Model file for the job. Use its own axes, mm. A direction names the side the tool comes from. Round coordinates to 2 decimals unless told otherwise and drop trailing zeros. Loops run counter-clockwise (first coordinate to the right, second up) from the corner with the lowest first, then second, coordinate; pieces in that order, holes last. Notation, with made-up numbers: M 61.5,46 L 92.5,46 A22 cw 92.5,54 Z; hole C 18.25,12.5 d4. An arc over 180 degrees is marked long. Answer in a Markdown table with one row per item.
from build123d import *

# Parameters (mm, degrees)
SKETCH1_R           = 40
BOSS_EXTRUDE1_DEPTH = 33
CUT_EXTRUDE1_START  = -6
SKETCH2_R           = 40
SKETCH2_R_2         = 38
CUT_EXTRUDE1_DEPTH  = 6
CHAMFER1_SIZE       = 5
SKETCH3_R           = 14
CUT_EXTRUDE2_DEPTH  = 13
CUT_EXTRUDE3_DEPTH  = 20


with BuildPart() as part:
    # Sketch1 → Boss-Extrude1 (new body)
    with BuildSketch(Plane.XY):
        Circle(SKETCH1_R)
    extrude(amount=BOSS_EXTRUDE1_DEPTH)

    # Sketch2 → Cut-Extrude1 (cut)
    with BuildSketch(Plane.XY.offset(33).offset(CUT_EXTRUDE1_START)):
        Circle(SKETCH2_R)
        Circle(SKETCH2_R_2, mode=Mode.SUBTRACT)
    extrude(amount=CUT_EXTRUDE1_DEPTH, mode=Mode.SUBTRACT)

    # Chamfer1
    chamfer1_edges = [part.edges().sort_by_distance(p)[0] for p in [
        (-40, 0, 0),
    ]]
    chamfer(chamfer1_edges, length=CHAMFER1_SIZE)

    # Sketch3 → Cut-Extrude2 (cut)
    with BuildSketch(Plane.XY.offset(33)):
        Circle(SKETCH3_R)
    extrude(amount=-CUT_EXTRUDE2_DEPTH, mode=Mode.SUBTRACT)

    # Sketch4 → Cut-Extrude3 (cut)
    with BuildSketch(Plane(origin=(0, 0, 0), x_dir=(-1, 0, 0), z_dir=(0, 0, -1))):
        Polygon((-19.5, -11.258330249), (0, -22.516660498), (19.5, -11.258330249), (19.5, 11.258330249), (0, 22.516660498), (-19.5, 11.258330249), align=None)
    extrude(amount=-CUT_EXTRUDE3_DEPTH, mode=Mode.SUBTRACT)


solid = part.part
1. Mould opens along X. For faces 4 (the flat face through (0, -15, 20)), 5 (the flat face through (35.4, -14.6, 27)), 6 (the cylindrical face through (12.932, -5.362, 26.591)), 7 (the cylindrical face through (-8.67, -39.05, 15.85)) say: +X half, -X half, draft (parallel to the pull), parting line (faces both ways), or undercut.
Verdict:
| item | result |
|---|---|
| face 4 | undercut |
| face 5 | draft |
| face 6 | undercut |
| face 7 | parting line |
2. Wall check: probe 1 along Y at (x, z) = (0, 26); probe 2 along X at (y, z) = (-21, 16); probe 3 along Y at (x, z) = (7.5, 13). Give the ranges that are in metal, low to high.
Verdict:
| item | result |
|---|---|
| probe 1 | y = -40 to -14, 14 to 40 |
| probe 2 | x = -34.04 to -2.63, 2.63 to 34.04 |
| probe 3 | y = -39.29 to -18.19, 18.19 to 39.29 |
3. Saw through at B-B (y = 0). Write the cut outline in (x, z), and give its area (3 significant figures).
Verdict:
| item | result |
|---|---|
| outline | M -40,5 L -35,0 L -19.5,0 L -19.5,20 L -14,20 L -14,33 L -38,33 L -38,27 L -40,27 Z; M 14,20 L 19.5,20 L 19.5,0 L 35,0 L 40,5 L 40,27 L 38,27 L 38,33 L 14,33 Z |
| area | 1,450 mm² |
4. Saw through at A-A (z = 7.5). Write the cut outline in (x, y).
Verdict:
| item | result |
|---|---|
| outline | C 0,0 d80; hole M -19.5,-11.26 L 0,-22.52 L 19.5,-11.26 L 19.5,11.26 L 0,22.52 L -19.5,11.26 Z |
5. Tool access for faces 1 (the cylindrical face through (17.535, -33.713, 29.958)), 2 (the flat face through (15, -15, 0)), 3 (the flat face through (9.61, 16.97, 9.86)): list every direction of +Z, -Z, +X, -X, +Y, -Y with a clear straight run to the whole face (end or side of a thin tool).
Verdict:
| item | result |
|---|---|
| face 1 | +Z |
| face 2 | -Z, +X, -X, +Y, -Y |
| face 3 | -Z |
6. Pin check, flat tips, straight feed: pin 1 (12 mm diameter, centred on x = 9, z = 19, fed in from -Y); pin 2 (10 mm diameter, centred on y = -18.5, z = 25.5, fed in from +X); pin 3 (1 mm diameter, centred on x = 5.5, z = 14.5, fed in from +Y); pin 4 (19.5 mm diameter, centred on x = -3, y = 1, fed in from -Z). Stop position of each tip, or through.
Verdict:
| item | result |
|---|---|
| pin 1 | stops at y = -39.89 |
| pin 2 | stops at x = 37.65 |
| pin 3 | stops at y = 39.69 |
| pin 4 | passes through |
7. Saw through at C-C (z = 22). Write the cut outline in (x, y).
Verdict:
| item | result |
|---|---|
| outline | C 0,0 d80; hole C 0,0 d28 |
